For this review, take the finished solid that the model builds, in its own axes (mm). A direction names the side the tool comes from. Coordinates: 2 decimals unless noted, no trailing zeros. Loops run counter-clockwise (first coordinate to the right, second up) from the corner with the lowest first, then second, coordinate; pieces in that order, holes last. Notation, with made-up numbers: (-23, 38) - (-11, 38) arc R22 ccw to (-11, 59) - close; hole circle Ø5 at (-18.5, 30.25). An arc over 180 degrees is marked (long way). Use one line per item in the form item = value. Start each with the question number.
1. Add section B-B on y = 86. Give the boundary of the cut face in (x, z), and give its area (3 significant figures).
2. To check wall thickness, follow probe 1 along Y at (x, z) = (-7, 2); probe 2 along Y at (x, z) = (30, 14.75); probe 3 along Y at (x, z) = (-117, 6.5). State the ranges of each line that lie inside material, in increasing order.
3. Add section C-C on z = 7. Count the separate pieces of the cut face and the enclosed holes in it, and give its area (3 significant figures).
4. Add section D-D on y = 274. Give the boundary of the cut face in (x, z).
5. Draft analysis for pull direction Y (two halves, no side actions). For faces 1 (the face through (-183.005, 384.346, 9.86)), 2 (the face through (150, 714, 10)), 3 (the face through (247.199, 443.254, 9.86)), 4 (the face through (-5.858, 494.617, 9.86)), state which applies: +Y half, -Y half, draft (parallel to the pull), parting line (faces both ways), or undercut.
6. For pin 1 Ø18.5 at (x, y) = (251.5, 450) entering from -Z; pin 2 Ø8 at (y, z) = (172.5, 9.5) entering from +X; pin 3 Ø3.5 at (x, z) = (152, 10) entering from -Y; pin 4 Ø10 at (y, z) = (263, 14.5) entering from -X, all flat-tipped, find the tip position at first contact; note any pin that passes through.
7. Machinability: for faces 5 (the face through (163, 699, 10)), 6 (the face through (150, 149, 10)), 7 (the face through (-150, 714, 10)), which of the approach directions +Z, -Z, +X, -X, +Y, -Y give a long, thin tool a straight path to every point of the face, cutting with its end or side? Answer none if there is none.
8. Add section A-A on x = 0. Give the boundary of the cut face in (y, z).
```python
from build123d import *

# Parameters (mm, degrees)
SKETCH1_R           = 45
SKETCH1_R_2         = 40
SKETCH1_R_3         = 8
BOSS_EXTRUDE1_DEPTH = 20
FILLET1_R           = 100
FILLET2_R           = 20
M10_TAPPED_HOLE1_D  = 8.5


with BuildPart() as part:
    # Sketch1 → Boss-Extrude1 (new body)
    with BuildSketch(Plane.XY):
        with BuildLine():
            Line((-150, 0), (150, 0))
            Line((150, 0), (150, 199))
            Line((150, 199), (153, 199))
            Line((153, 199), (153, 302))
            ThreePointArc((153, 302), (190.490332008, 392.509667992), (281, 430))
            Line((281, 430), (175, 699))
            Line((175, 699), (150, 699))
            Line((150, 699), (150, 729))
            Line((150, 729), (-150, 729))
            Line((-150, 729), (-150, 699))
            Line((-150, 699), (-175, 699))
            Line((-175, 699), (-281, 430))
            ThreePointArc((-281, 430), (-190.490332008, 392.509667992), (-153, 302))
            Line((-153, 302), (-153, 199))
            Line((-153, 199), (-150, 199))
            Line((-150, 199), (-150, 0))
        make_face()
        with Locations((0, 450)):
            Circle(SKETCH1_R, mode=Mode.SUBTRACT)
        with Locations((0, 70)):
            Circle(SKETCH1_R_2, mode=Mode.SUBTRACT)
        with Locations((-251.5, 450)):
            Circle(SKETCH1_R_3, mode=Mode.SUBTRACT)
        with Locations(Location((251.5, 450, 0), (0, 0, 180))):
            Circle(SKETCH1_R_3, mode=Mode.SUBTRACT)
    extrude(amount=BOSS_EXTRUDE1_DEPTH)

    # Fillet1
    fillet1_edges = [part.edges().sort_by_distance(p)[0] for p in [
        (150, 0, 10),
        (-150, 0, 10),
    ]]
    fillet(fillet1_edges, radius=FILLET1_R)

    # Fillet2
    fillet2_edges = [part.edges().sort_by_distance(p)[0] for p in [
        (-281, 430, 10),
        (281, 430, 10),
    ]]
    fillet(fillet2_edges, radius=FILLET2_R)

    # M10 Tapped Hole1 (through all)
    with Locations(Plane.XY.offset(20)):
        with Locations((-30, 370), (-30, 142), (30, 142), (30, 370)):
            Hole(M10_TAPPED_HOLE1_D / 2)


solid = part.part
```
Conclusion:
q1.outline = (-149.02, 0) - (-36.66, 0) - (-36.66, 20) - (-149.02, 20) - close; (36.66, 0) - (149.02, 0) - (149.02, 20) - (36.66, 20) - close
q1.area = 4,490 mm^2
q2.probe_1 = 0 to 30.62, 109.38 to 405.55, 494.45 to 729
q2.probe_2 = 0 to 43.54, 96.46 to 137.75, 146.25 to 365.75, 374.25 to 416.46, 483.54 to 729
q2.probe_3 = 25.76 to 729
q3.separate_pieces = 1
q3.enclosed_holes = 8
q3.area = 252,000 mm^2
q4.outline = (-153, 0) - (153, 0) - (153, 20) - (-153, 20) - close
q5.face_1 = -Y half
q5.face_2 = draft
q5.face_3 = undercut
q5.face_4 = undercut
q6.pin_1 = 0
q6.pin_2 = 150
q6.pin_3 = 199
q6.pin_4 = -153
q7.face_5 = +Z, -Z, +X, +Y
q7.face_6 = +Z, -Z, +X, -Y
q7.face_7 = +Z, -Z, -X, +Y
q8.outline = (0, 0) - (30, 0) - (30, 20) - (0, 20) - close; (110, 0) - (405, 0) - (405, 20) - (110, 20) - close; (495, 0) - (729, 0) - (729, 20) - (495, 20) - close
